Build history of the part. All positions in model axes, mm. Round coordinates to 2 decimals unless told otherwise and drop trailing zeros. Write each loop counter-clockwise with the first axis right and the second up, starting at its lowest first coordinate (ties: lowest second). Pieces come first, ordered by that corner, then holes.
Item 1: Mould opens along Z. For faces 1 (the flat face through (-1, 12, -60)), 2 (the flat face through (-1, 12, 60)), 3 (the cylindrical face through (25.553, 11.832, 33.286)), 4 (the cylindrical face through (25.553, 11.832, -41.714)) say: +Z half, -Z half, draft (parallel to the pull), parting line (faces both ways), or undercut.
Item 2: Band-saw the part on C-C, the plane z = -37.5. Write the cut outline in (x, y).
Item 3: Band-saw the part on B-B, the plane y = 18.25. Write the cut outline in (x, z), then the cut area to 3 significant figures.
Item 4: Band-saw the part on A-A, the plane x = -25. Write the cut outline in (y, z), then the cut area to 3 significant figures.
Item 5: Wall check: probe 1 along X at (y, z) = (11, -37.5); probe 2 along Z at (x, y) = (-25, 16.75); probe 3 along Z at (x, y) = (-21.5, 2.5). Give the ranges that are in metal, low to high.
```python
from build123d import *

# Parameters (mm, degrees)
SKETCH_1_W          = 90
SKETCH_1_H          = 120
EXTRUDE_1_DEPTH     = 24
HOLE_WIZARD_M10_1_D = 8.5


with BuildPart() as part:
    # 草图1 → 凸台-拉伸1 (new body)
    with BuildSketch(Plane(origin=(0, 0, 0), x_dir=(1, 0, 0), z_dir=(0, 1, 0))):
        Rectangle(SKETCH_1_W, SKETCH_1_H)
    extrude(amount=EXTRUDE_1_DEPTH)

    # M10 螺纹孔1 (through all)
    with Locations(Plane(origin=(0, 24, 0), x_dir=(1, 0, 0), z_dir=(0, 1, 0))):
        with Locations((-25, -37.5), (-25, 37.5), (25, 37.5), (25, -37.5)):
            Hole(HOLE_WIZARD_M10_1_D / 2)


solid = part.part
```
Results:
1. face 1: -Z half
1. face 2: +Z half
1. face 3: undercut
1. face 4: undercut
2. outline: (-45, 0) - (-29.25, 0) - (-29.25, 24) - (-45, 24) - close; (-20.75, 0) - (20.75, 0) - (20.75, 24) - (-20.75, 24) - close; (29.25, 0) - (45, 0) - (45, 24) - (29.25, 24) - close
3. outline: (-45, -60) - (45, -60) - (45, 60) - (-45, 60) - close; hole circle Ø8.5 at (-25, -37.5); hole circle Ø8.5 at (-25, 37.5); hole circle Ø8.5 at (25, -37.5); hole circle Ø8.5 at (25, 37.5)
3. area: 10,600 mm2
4. outline: (0, -60) - (24, -60) - (24, -41.75) - (0, -41.75) - close; (0, -33.25) - (24, -33.25) - (24, 33.25) - (0, 33.25) - close; (0, 41.75) - (24, 41.75) - (24, 60) - (0, 60) - close
4. area: 2,470 mm2
5. probe 1: x = -45 to -29.25, -20.75 to 20.75, 29.25 to 45
5. probe 2: z = -60 to -41.75, -33.25 to 33.25, 41.75 to 60
5. probe 3: z = -60 to -39.91, -35.09 to 35.09, 39.91 to 60
